```python
from build123d import *

# Parameters (mm, degrees)
SKETCH1_W           = 75
SKETCH1_H           = 20
SKETCH1_R           = 2.5
BOSS_EXTRUDE1_DEPTH = 3
FILLET1_R           = 5


with BuildPart() as part:
    # Sketch1 → Boss-Extrude1 (new body)
    with BuildSketch(Plane.XY):
        with Locations((37.5, -10)):
            Rectangle(SKETCH1_W, SKETCH1_H)
        with Locations((10, -10)):
            Circle(SKETCH1_R, mode=Mode.SUBTRACT)
        with Locations((65, -10)):
            Circle(SKETCH1_R, mode=Mode.SUBTRACT)
        with Locations((37.5, -10)):
            Circle(SKETCH1_R, mode=Mode.SUBTRACT)
    extrude(amount=BOSS_EXTRUDE1_DEPTH)

    # Fillet1
    fillet1_edges = [part.edges().sort_by_distance(p)[0] for p in [
        (0, 0, 1.5),
        (75, 0, 1.5),
    ]]
    fillet(fillet1_edges, radius=FILLET1_R)


solid = part.part
```
For this review, take the finished solid that the model builds, in its own axes (mm). Round coordinates to 2 decimals unless told otherwise and drop trailing zeros. Write each loop counter-clockwise with the first axis right and the second up, starting at its lowest first coordinate (ties: lowest second). Pieces come first, ordered by that corner, then holes. Notation, with made-up numbers: (-39.75, -25) -> (-9.75, -25) arc R33 ccw to (-9.75, 8) -> close; hole circle Ø9 at (-13, 57.5). An arc over 180 degrees is marked (long way). One line per question, with ' | ' between items. Start each with the question number.
1) Add section B-B (x = 10). Write out the cut boundary in (y, z), and give its area (3 significant figures).
2) Wall thickness on line 1 along X through (y, z) = (-9.75, 1.95); line 2 along Y through (x, z) = (10, 2.2); line 3 along X through (y, z) = (-11.75, 0.6): over which ranges is each line inside the solid? List them lowest first.
3) Add section A-A (z = 0.9). Write out the cut boundary in (x, y).
4) Add section C-C (y = -9). Write out the cut boundary in (x, z), and give its area (3 significant figures).
5) Mouldability with a two-part tool opening along Y and no side actions: class faces 1 (the cylindrical face through (39.81, -10.96, 1.48)), 2 (the flat face through (75, -13, 1)), 3 (the cylindrical face through (1, -2, 2)) as +Y half, -Y half, draft (parallel to the pull), parting line (faces both ways), or undercut.
6) For pin 1 Ø8 at (x, y) = (65, -10) entering from +Z; pin 2 Ø4 at (x, y) = (37.5, -10) entering from +Z, all flat-tipped, find the tip position at first contact; note any pin that passes through.
7) Add section D-D (y = -2). Write out the cut boundary in (x, z), and give its area (3 significant figures).
Reported:
1) outline: (-20, 0) -> (-12.5, 0) -> (-12.5, 3) -> (-20, 3) -> close; (-7.5, 0) -> (0, 0) -> (0, 3) -> (-7.5, 3) -> close | area: 45.0 mm²
2) line 1: x = 0 to 7.51, 12.49 to 35.01, 39.99 to 62.51, 67.49 to 75 | line 2: y = -20 to -12.5, -7.5 to 0 | line 3: x = 0 to 8.21, 11.79 to 35.71, 39.29 to 63.21, 66.79 to 75
3) outline: (0, -20) -> (75, -20) -> (75, -5) arc R5 ccw to (70, 0) -> (5, 0) arc R5 ccw to (0, -5) -> close; hole circle Ø5 at (10, -10); hole circle Ø5 at (37.5, -10); hole circle Ø5 at (65, -10)
4) outline: (0, 0) -> (7.71, 0) -> (7.71, 3) -> (0, 3) -> close; (12.29, 0) -> (35.21, 0) -> (35.21, 3) -> (12.29, 3) -> close; (39.79, 0) -> (62.71, 0) -> (62.71, 3) -> (39.79, 3) -> close; (67.29, 0) -> (75, 0) -> (75, 3) -> (67.29, 3) -> close | area: 184 mm²
5) face 1: undercut | face 2: draft | face 3: +Y half
6) pin 1: stops at z = 3 | pin 2: passes through
7) outline: (1, 0) -> (74, 0) -> (74, 3) -> (1, 3) -> close | area: 219 mm²
